from build123d import *

# Parameters (mm, degrees)
SKETCH_1_W      = 180
SKETCH_1_H      = 60
EXTRUDE_1_DEPTH = 10


with BuildPart() as part:
    # 草图1 → 凸台-拉伸1 (new body)
    with BuildSketch(Plane.XY):
        Rectangle(SKETCH_1_W, SKETCH_1_H)
        with BuildLine():
            Line((-71.5, 21), (-63.5, 21))
            ThreePointArc((-63.5, 21), (-57.5, 15), (-63.5, 9))
            Line((-63.5, 9), (-71.5, 9))
            ThreePointArc((-71.5, 9), (-77.5, 15), (-71.5, 21))
        make_face(mode=Mode.SUBTRACT)
        with BuildLine():
            Line((63.5, 21), (71.5, 21))
            ThreePointArc((71.5, 21), (77.5, 15), (71.5, 9))
            Line((71.5, 9), (63.5, 9))
            ThreePointArc((63.5, 9), (57.5, 15), (63.5, 21))
        make_face(mode=Mode.SUBTRACT)
    extrude(amount=EXTRUDE_1_DEPTH)


solid = part.part
Read the model definition and answer for the solid it produces. Units are mm, in the model's axes. A direction names the side the tool comes from. Round coordinates to 2 decimals unless told otherwise and drop trailing zeros. Write each loop counter-clockwise with the first axis right and the second up, starting at its lowest first coordinate (ties: lowest second). Pieces come first, ordered by that corner, then holes. Notation, with made-up numbers: (-15, -40) - (27, -40) arc R26 ccw to (27, -13) - close; hole circle Ø8 at (-39, 60). An arc over 180 degrees is marked (long way). Use a Markdown table: item, result.
(1) Which of the six approach directions +Z, -Z, +X, -X, +Y, -Y give full straight-line access (tool end or side, diameter ignored) to faces 1 (the cylindrical face through (-77.5, 14.9, 4.9)), 2 (the flat face through (-1, 0, 0))?
Reported:
| item | result |
|---|---|
| face 1 | +Z, -Z |
| face 2 | -Z, +X, -X, +Y, -Y |
(2) The part is cut by section C-C (z = 2.75). Write down the section's boundary in (x, y).
Reported:
| item | result |
|---|---|
| outline | (-90, -30) - (90, -30) - (90, 30) - (-90, 30) - close; hole (-71.5, 9) - (-63.5, 9) arc R6 ccw to (-63.5, 21) - (-71.5, 21) arc R6 ccw to start; hole (63.5, 9) - (71.5, 9) arc R6 ccw to (71.5, 21) - (63.5, 21) arc R6 ccw to start |
(3) Straight lines are drawn through the part: line 1 along Y through (x, z) = (-72, 1.5); line 2 along X through (y, z) = (17, 2.75); line 3 along X through (y, z) = (17.5, 7.25). For each, find the intervals that lie inside material, in ascending order. Write a range as [from, to].
Reported:
| item | result |
|---|---|
| line 1 | [-30, 9.02], [20.98, 30] |
| line 2 | [-90, -77.16], [-57.84, 57.84], [77.16, 90] |
| line 3 | [-90, -76.95], [-58.05, 58.05], [76.95, 90] |
(4) The part is cut by section B-B (x = -69). Write down the section's boundary in (y, z), then the cut area to 3 significant figures.
Reported:
| item | result |
|---|---|
| outline | (-30, 0) - (9, 0) - (9, 10) - (-30, 10) - close; (21, 0) - (30, 0) - (30, 10) - (21, 10) - close |
| area | 480 mm2 |
(5) The mould has two halves that part along X. Classify faces 3 (the flat face through (-1, 30, 5)), 4 (the flat face through (-90, 0, 5)), 5 (the flat face through (67, 21, 5)), 6 (the flat face through (90, 0, 5)): released by +X, released by -X, zero draft, split by the parting line, or undercut.
Reported:
| item | result |
|---|---|
| face 3 | zero draft |
| face 4 | released by -X |
| face 5 | undercut |
| face 6 | released by +X |
(6) The part is cut by section A-A (y = 15). Write down the section's boundary in (x, z).
Reported:
| item | result |
|---|---|
| outline | (-90, 0) - (-77.5, 0) - (-77.5, 10) - (-90, 10) - close; (-57.5, 0) - (57.5, 0) - (57.5, 10) - (-57.5, 10) - close; (77.5, 0) - (90, 0) - (90, 10) - (77.5, 10) - close |
(7) This flat-tipped pin is pushed along its axis until it touches: pin 1 Ø5 at (x, y) = (36, 16) entering from -Z. Where does it stop, or does it pass through?
Reported:
| item | result |
|---|---|
| pin 1 | z = 0 |
